```python
from build123d import *

# Parameters (mm, degrees)
BOSS_EXTRUDE1_DEPTH = 2000
SKETCH2_R           = 6
CUT_EXTRUDE1_DEPTH  = 2002.278667491
SKETCH3_R           = 3.25
BOSS_EXTRUDE2_DEPTH = 10


with BuildPart() as part:
    # Sketch1 → Boss-Extrude1 (new body)
    with BuildSketch(Plane.XY):
        with BuildLine():
            Line((-2.78812886, -2.868159246), (-2.78812886, -59.687153545))
            ThreePointArc((-2.78812886, -59.687153545), (0.061942892, -70.999680248), (2.677842692, -59.630720857))
            Line((2.677842692, -59.630720857), (2.677842692, -2.971389998))
            ThreePointArc((2.677842692, -2.971389998), (0.075530833, 3.999286823), (-2.78812886, -2.868159246))
        make_face()
    extrude(amount=BOSS_EXTRUDE1_DEPTH)

    # Sketch2 → Cut-Extrude1 (cut, through all)
    with BuildSketch(Plane(origin=(2.677842692, 0, 0), x_dir=(0, 0, -1), z_dir=(1, 0, 0))):
        with Locations(Location((-200, -14.971389998, 0), (0, 0, 90))):
            Circle(SKETCH2_R)
        with Locations(Location((-600, -14.971389998, 0), (0, 0, 90))):
            Circle(SKETCH2_R)
        with Locations(Location((-1000, -14.971389998, 0), (0, 0, 90))):
            Circle(SKETCH2_R)
        with Locations(Location((-1400, -14.971389998, 0), (0, 0, 90))):
            Circle(SKETCH2_R)
        with Locations(Location((-1800, -14.971389998, 0), (0, 0, 90))):
            Circle(SKETCH2_R)
    extrude(amount=-CUT_EXTRUDE1_DEPTH, mode=Mode.SUBTRACT)

    # Sketch3 → Boss-Extrude2 (add)
    with BuildSketch(Plane(origin=(0, 0, 0), x_dir=(1, 0, 0), z_dir=(0, 1, 0))):
        with Locations(Location((0, -200, 0), (0, 0, 90))):
            Circle(SKETCH3_R)
        with Locations(Location((0, -1800, 0), (0, 0, 90))):
            Circle(SKETCH3_R)
    extrude(amount=BOSS_EXTRUDE2_DEPTH)


solid = part.part
```
For this review, take the finished solid that the model builds, in its own axes (mm). A direction names the side the tool comes from. Give positions to 0.01 mm unless a question says otherwise; leave off trailing zeros. Order: outer loops, then holes, each group sorted by start corner. A loop starts at its lowest first (then second) coordinate and runs counter-clockwise, first axis right, second up.
1) Take a section at A-A (x = 0). Give the boundary of the cut face in (y, z), then the cut area to 3 significant figures.
2) Wall thickness on line 1 (Y direction, x = -1.05, z = 600); line 2 (Y direction, x = 0.45, z = 1800); line 3 (X direction, y = -55, z = 1887.5): over which ranges is each line inside the solid? List them lowest first.
3) Take a section at C-C (y = -44). Give the boundary of the cut face in (x, z).
4) Take a section at B-B (z = 1608). Give the boundary of the cut face in (x, y), then the cut area to 3 significant figures.
5) For faces 1 (the face through (2.678, -32, 986)), 2 (the face through (-2.788, -31, 986)), list the 3-axis set-ups (+Z, -Z, +X, -X, +Y, -Y) from which the entire face can be reached by the end or side of a thin tool; tool diameter is ignored.
6) Insertion check: pin 1 (17 mm diameter, centred on y = -33, z = 796.5, fed in from +X); pin 2 (2 mm diameter, centred on y = -50.5, z = 450, fed in from -X); pin 3 (4 mm diameter, centred on x = 4.5, z = 841, fed in from +Y). Each pin has a flat end and moves straight along its axis. Give the tip position at first contact, or say it passes through.
Derived:
1. outline: (-71, 0) - (4, 0) - (4, 196.75) - (10, 196.75) - (10, 203.25) - (4, 203.25) - (4, 1796.75) - (10, 1796.75) - (10, 1803.25) - (4, 1803.25) - (4, 2000) - (-71, 2000) - close; hole circle Ø12 at (-14.97, 200); hole circle Ø12 at (-14.97, 600); hole circle Ø12 at (-14.97, 1000); hole circle Ø12 at (-14.97, 1400); hole circle Ø12 at (-14.97, 1800)
1. area: 150,000 mm2
2. line 1: y = -70.91 to -20.97, -8.97 to 3.86
2. line 2: y = -70.98 to -20.97, -8.97 to 10
2. line 3: x = -2.79 to 2.68
3. outline: (-2.79, 0) - (2.68, 0) - (2.68, 2000) - (-2.79, 2000) - close
4. outline: (-2.79, -59.69) arc R6 ccw (long way) to (2.68, -59.63) - (2.68, -2.97) arc R4 ccw (long way) to (-2.79, -2.87) - close
4. area: 467 mm2
5. face 1: +Z, -Z, +X
5. face 2: +Z, -Z, -X
6. pin 1: stops at x = 2.68
6. pin 2: stops at x = -2.79
6. pin 3: stops at y = 3.12
